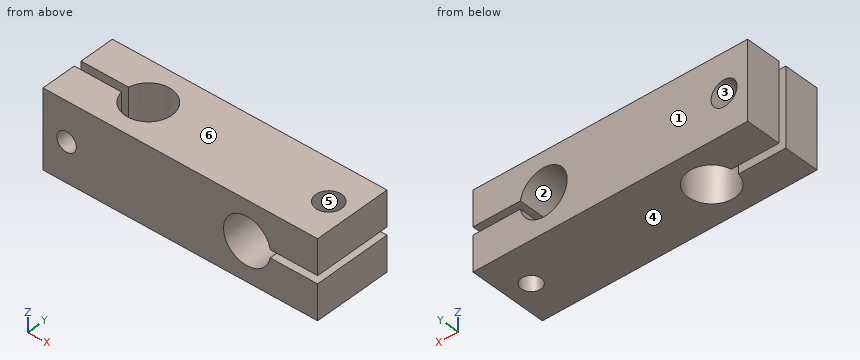
from build123d import *

# Parameters (mm, degrees)
SKETCH1_R             = 2
BOSS_EXTRUDE1_DEPTH   = 20
HOLE1_D               = 6.6
HOLE1_DEPTH           = 9
M6_TAPPED_HOLE1_D     = 5
M6_TAPPED_HOLE1_DEPTH = 9
M6_TAPPED_HOLE1_TIP   = 1.502151548
SKETCH6_R             = 2
CUT_EXTRUDE1_DEPTH    = 51.206971578
M6_TAPPED_HOLE2_D     = 5
M6_TAPPED_HOLE2_DEPTH = 9
M6_TAPPED_HOLE2_TIP   = 1.502151548
HOLE2_D               = 6.6
HOLE2_DEPTH           = 9


with BuildPart() as part:
    # Sketch1 → Boss-Extrude1 (new body)
    with BuildSketch(Plane.XY):
        with BuildLine():
            Line((-41.48180318, 24.678559646), (28.51819682, 24.678559646))
            Line((28.51819682, 24.678559646), (28.51819682, 4.678559646))
            Line((28.51819682, 4.678559646), (-41.48180318, 4.678559646))
            Line((-41.48180318, 4.678559646), (-41.48180318, 13.678559646))
            Line((-41.48180318, 13.678559646), (-29.397882963, 13.678559646))
            ThreePointArc((-29.397882963, 13.678559646), (-17.48180318, 14.678559646), (-29.397882963, 15.678559646))
            Line((-29.397882963, 15.678559646), (-41.48180318, 15.678559646))
            Line((-41.48180318, 15.678559646), (-41.48180318, 24.678559646))
        make_face()
        with Locations((22.51819682, 14.678559646)):
            Circle(SKETCH1_R, mode=Mode.SUBTRACT)
    extrude(amount=BOSS_EXTRUDE1_DEPTH)

    # Hole1
    with Locations(Plane.XY.offset(20)):
        with Locations((22.51819682, 14.678559646)):
            Hole(HOLE1_D / 2, depth=HOLE1_DEPTH)

    # M6 Tapped Hole1
    with Locations(Plane(origin=(0, 0, 0), x_dir=(-1, 0, 0), z_dir=(0, 0, -1))):
        with Locations((-22.51819682, 14.678559646)):
            Hole(M6_TAPPED_HOLE1_D / 2, depth=M6_TAPPED_HOLE1_DEPTH)
            with Locations((0, 0, -(M6_TAPPED_HOLE1_DEPTH + M6_TAPPED_HOLE1_TIP / 2))):  # 118° drill point
                Cone(0, M6_TAPPED_HOLE1_D / 2, M6_TAPPED_HOLE1_TIP, mode=Mode.SUBTRACT)

    # Sketch6 → Cut-Extrude1 (cut, through all)
    with BuildSketch(Plane(origin=(0, 24.678559646, 0), x_dir=(1, 0, 0), z_dir=(0, 1, 0))):
        with Locations(Location((-35.48180318, -10, 0), (0, 0, 270))):
            Circle(SKETCH6_R)
        with BuildLine():
            Line((16.434276603, -11), (30.650689968, -11))
            Line((30.650689968, -11), (30.650689968, -9))
            Line((30.650689968, -9), (16.434276603, -9))
            ThreePointArc((16.434276603, -9), (4.51819682, -10), (16.434276603, -11))
        make_face()
    extrude(amount=-CUT_EXTRUDE1_DEPTH, mode=Mode.SUBTRACT)

    # M6 Tapped Hole2
    with Locations(Plane(origin=(0, 4.678559646, 0), x_dir=(-1, 0, 0), z_dir=(0, -1, 0))):
        with Locations((35.48180318, -10)):
            Hole(M6_TAPPED_HOLE2_D / 2, depth=M6_TAPPED_HOLE2_DEPTH)
            with Locations((0, 0, -(M6_TAPPED_HOLE2_DEPTH + M6_TAPPED_HOLE2_TIP / 2))):  # 118° drill point
                Cone(0, M6_TAPPED_HOLE2_D / 2, M6_TAPPED_HOLE2_TIP, mode=Mode.SUBTRACT)

    # Hole2
    with Locations(Plane(origin=(0, 24.678559646, 0), x_dir=(1, 0, 0), z_dir=(0, 1, 0))):
        with Locations((-35.48180318, -10)):
            Hole(HOLE2_D / 2, depth=HOLE2_DEPTH)


solid = part.part
Geometry: final body of the model. Coordinates: model frame, mm. Face numbers are marked on the shaded views. A direction names the side the tool comes from. Coordinates: 2 decimals unless noted, no trailing zeros. Order: outer loops, then holes, each group sorted by start corner. A loop starts at its lowest first (then second) coordinate and runs counter-clockwise, first axis right, second up.
(1) Section query A-A (z = 10). Return the cut outline in (x, y), plus the area to 3 significant figures.
(2) Section query B-B (x = 9). Return the cut outline in (y, z).
(3) Section query D-D (z = 17.5). Return the cut outline in (x, y).
(4) Section query C-C (y = 6.5). Return the cut outline in (x, z), plus the area to 3 significant figures.
(5) Draft query along Z for the marked faces 1, 2, 3 and 4. Return one class per face: pulls with the +Z half, pulls with the -Z half, needs draft (parallel to the pull), parting line crosses it, or undercut.
(6) First-contact query: pin 1 (7 mm diameter, centred on x = -23.48, y = 14.68, fed in from -Z); pin 2 (6 mm diameter, centred on x = 22.5, y = 14.5, fed in from +Z). Flat tips, straight axial feed; report the tip coordinate or a pass-through.
(7) Material intervals for probe 1 along X at (y, z) = (18.5, 6); probe 2 along Y at (x, z) = (-31, 11); probe 3 along Z at (x, y) = (10.5, 10), sorted ascending.
(8) Access query for the marked faces 5 and 6. Directions: +Z, -Z, +X, -X, +Y, -Y. A direction counts if a zero-diameter tool reaches every point of the face in a straight line with its end or side. Return the directions, or none.
Solution:
1. outline: (-41.48, 4.68) - (-37.98, 4.68) - (-37.98, 13.68) - (-41.48, 13.68) - close; (-41.48, 15.68) - (-38.78, 15.68) - (-38.78, 24.68) - (-41.48, 24.68) - close; (-32.98, 4.68) - (4.52, 4.68) - (4.52, 24.68) - (-32.18, 24.68) - (-32.18, 15.68) - (-29.4, 15.68) arc R6 cw (long way) to (-29.4, 13.68) - (-32.98, 13.68) - close
1. area: 678 mm2
2. outline: (4.68, 0) - (24.68, 0) - (24.68, 4.2) - (4.68, 4.2) - close; (4.68, 15.8) - (24.68, 15.8) - (24.68, 20) - (4.68, 20) - close
3. outline: (-41.48, 4.68) - (28.52, 4.68) - (28.52, 24.68) - (-41.48, 24.68) - (-41.48, 15.68) - (-29.4, 15.68) arc R6 cw (long way) to (-29.4, 13.68) - (-41.48, 13.68) - close; hole circle Ø6.6 at (22.52, 14.68)
4. outline: (-41.48, 0) - (28.52, 0) - (28.52, 9) - (16.43, 9) arc R6 cw (long way) to (16.43, 11) - (28.52, 11) - (28.52, 20) - (-41.48, 20) - close; hole circle Ø5 at (-35.48, 10)
4. area: 1,240 mm2
5. face 1: needs draft
5. face 2: undercut
5. face 3: undercut
5. face 4: pulls with the -Z half
6. pin 1: passes through
6. pin 2: stops at z = 9
7. probe 1: x = -41.48 to -28.11, -18.86 to 6.05, 14.99 to 28.52
7. probe 2: y = 4.68 to 13.68, 15.68 to 24.68
7. probe 3: z = 0 to 4, 16 to 20
8. face 5: +Z
8. face 6: +Z, +X, -X, +Y, -Y
